Work out the finished part from the listing and answer in its coordinate system (mm). Round coordinates to 2 decimals unless told otherwise and drop trailing zeros. Write each loop counter-clockwise with the first axis right and the second up, starting at its lowest first coordinate (ties: lowest second). Pieces come first, ordered by that corner, then holes. Notation, with made-up numbers: M 25,-28 L 67,-28 A17 ccw 67,-6 Z; hole C 87,20.25 d11. An arc over 180 degrees is marked long. One line per item, written item: value. Start each with the question number.
Q1. Find section A-A (x = 90). Write down the section's boundary in (y, z).
Q2. Given pin 1 Ø0.9 at (y, z) = (478, 2) entering from +X, flat-ended and moving along its own axis, determine where the tip first touches the part or whether it passes through.
Q3. Consider probe 1 along Y at (x, z) = (90, 1.35); probe 2 along X at (y, z) = (461, 1.65). Determine where each line is inside the solid, lowest interval first.
Q4. The mould has two halves that part along Y. Classify faces 1 (the cylindrical face through (97.81, 564.49, 1.48)), 2 (the flat face through (261, 591, 3)): released by +Y, released by -Y, zero draft, split by the parting line, or undercut.
Q5. Find section C-C (z = 2.3). Write down the section's boundary in (x, y).
Q6. Find section B-B (y = 505). Write down the section's boundary in (x, z).
from build123d import *

# Parameters (mm, degrees)
SKETCH1_W           = 530
SKETCH1_H           = 1165
BOSS_EXTRUDE1_DEPTH = 3
SKETCH2_R           = 60
SKETCH2_W           = 120
SKETCH2_H           = 120
CUT_EXTRUDE1_DEPTH  = 10


with BuildPart() as part:
    # Sketch1 → Boss-Extrude1 (new body)
    with BuildSketch(Plane.XY):
        with Locations((265, 582.5)):
            Rectangle(SKETCH1_W, SKETCH1_H)
    extrude(amount=BOSS_EXTRUDE1_DEPTH)

    # Sketch2 → Cut-Extrude1 (cut)
    with BuildSketch(Plane(origin=(0, 0, 0), x_dir=(-1, 0, 0), z_dir=(0, 0, -1))):
        with Locations((-90, 505)):
            Circle(SKETCH2_R)
        with Locations((-490, 505)):
            Rectangle(SKETCH2_W, SKETCH2_H)
    extrude(amount=-CUT_EXTRUDE1_DEPTH, mode=Mode.SUBTRACT)


solid = part.part
The answers:
1. outline: M 0,0 L 445,0 L 445,3 L 0,3 Z; M 565,0 L 1165,0 L 1165,3 L 565,3 Z
2. pin 1: x = 430
3. probe 1: 0 to 445, 565 to 1165
3. probe 2: 0 to 49.21, 130.79 to 430
4. face 1: undercut
4. face 2: zero draft
5. outline: M 0,0 L 530,0 L 530,445 L 430,445 L 430,565 L 530,565 L 530,1165 L 0,1165 Z; hole C 90,505 d120
6. outline: M 0,0 L 30,0 L 30,3 L 0,3 Z; M 150,0 L 430,0 L 430,3 L 150,3 Z
